```python
from build123d import *

# Parameters (mm, degrees)
SKETCH1_W           = 40
SKETCH1_H           = 40
BOSS_EXTRUDE1_DEPTH = 10
BOSS_EXTRUDE2_DEPTH = 5
SKETCH4_R           = 5
CUT_EXTRUDE1_DEPTH  = 52.5


with BuildPart() as part:
    # Sketch1 → Boss-Extrude1 (new body)
    with BuildSketch(Plane(origin=(0, 0, 0), x_dir=(1, 0, 0), z_dir=(0, 1, 0))):
        Rectangle(SKETCH1_W, SKETCH1_H)
    extrude(amount=BOSS_EXTRUDE1_DEPTH)

    # Sketch2 → Boss-Extrude2 (add)
    with BuildSketch(Plane(origin=(20, 0, 0), x_dir=(0, 0, -1), z_dir=(1, 0, 0))):
        with BuildLine():
            Line((-20, 10), (-20, 25))
            ThreePointArc((-20, 25), (0, 45), (20, 25))
            Line((20, 25), (20, 10))
            Line((20, 10), (-20, 10))
        make_face()
    boss_extrude2 = extrude(amount=-BOSS_EXTRUDE2_DEPTH)

    # Mirror1: Boss-Extrude2 across plane
    add(boss_extrude2.mirror(Plane(origin=(0, 0, 0), x_dir=(0, 0, 1), z_dir=(1, 0, 0))))

    # Sketch4 → Cut-Extrude1 (cut, symmetric)
    with BuildSketch(Plane(origin=(17.5, 0, 0), x_dir=(0, 0, -1), z_dir=(1, 0, 0))):
        with Locations((0, 25)):
            Circle(SKETCH4_R)
    extrude(amount=CUT_EXTRUDE1_DEPTH, both=True, mode=Mode.SUBTRACT)


solid = part.part
```
Geometry check sheet. Reference: the model listing, model coordinates, mm. A direction names the side the tool comes from. Coordinates: 2 decimals unless noted, no trailing zeros. Order: outer loops, then holes, each group sorted by start corner. A loop starts at its lowest first (then second) coordinate and runs counter-clockwise, first axis right, second up. Notation, with made-up numbers: (7, 10) - (59, 10) arc R23 cw to (59, 21) - close; hole circle Ø1 at (45.25, 1). An arc over 180 degrees is marked (long way). Answer as a JSON object with one key per item and string values. Group by question number.
Item 1: Tool access check on faces 1 (the face through (0, 7, 20)), 2 (the face through (-15, 28, -5)). Record the directions out of +Z, -Z, +X, -X, +Y, -Y that give a thin tool (end or side, any length) a straight path to the whole face; none if there is none.
Item 2: Draft check along X on faces 3 (the face through (20, 18, 0)), 4 (the face through (0, 10, 0)), 5 (the face through (15, 28, -5)), 6 (the face through (0, 0, 0)). Enter one of: +X half, -X half, draft (parallel to the pull), parting line (faces both ways), or undercut.
Item 3: Sectioned sample at B-B, the plane x = 17.5. Record the cut outline in (y, z).
Item 4: Sectioned sample at D-D, the plane x = 3. Record the cut outline in (y, z), and give its area (3 significant figures).
Item 5: Sectioned sample at C-C, the plane z = 11.5. Record the cut outline in (x, y).
Item 6: Scan lines: probe 1 along X at (y, z) = (33.5, 10); probe 2 along Y at (x, z) = (17.5, 0); probe 3 along Y at (x, z) = (-13.5, 2). Record each from-to range of solid material in increasing order.
Item 7: Depth check by flat-ended pin: pin 1 Ø10 at (x, y) = (14, 30.5) entering from -Z; pin 2 Ø4 at (x, z) = (3.5, -7) entering from +Y. Enter the tip coordinate at first touch or a pass-through.
Item 8: Sectioned sample at A-A, the plane z = 0. Record the cut outline in (x, y), and give its area (3 significant figures).
Resolved:
{
 "1": {"face 1": "+Z, +X, -X, +Y, -Y", "face 2": "+Z, -Z, +Y"},
 "2": {"face 3": "+X half", "face 4": "undercut", "face 5": "undercut", "face 6": "draft"},
 "3": {"outline": "(0, -20) - (25, -20) arc R20 ccw to (25, 20) - (0, 20) - close; hole circle Ø10 at (25, 0)"},
 "4": {"outline": "(0, -20) - (10, -20) - (10, 20) - (0, 20) - close", "area": "400 mm^2"},
 "5": {"outline": "(-20, 0) - (20, 0) - (20, 41.36) - (15, 41.36) - (15, 10) - (-15, 10) - (-15, 41.36) - (-20, 41.36) - close"},
 "6": {"probe 1": "-20 to -15, 15 to 20", "probe 2": "0 to 20, 30 to 45", "probe 3": "0 to 10"},
 "7": {"pin 1": "z = -19.99", "pin 2": "y = 10"},
 "8": {"outline": "(-20, 0) - (20, 0) - (20, 20) - (15, 20) - (15, 10) - (-15, 10) - (-15, 20) - (-20, 20) - close; (-20, 30) - (-15, 30) - (-15, 45) - (-20, 45) - close; (15, 30) - (20, 30) - (20, 45) - (15, 45) - close", "area": "650 mm^2"}
}
